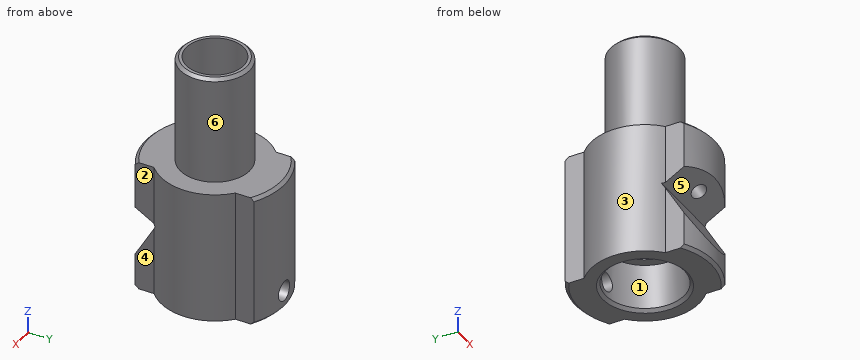
from build123d import *

# Parameters (mm, degrees)
SKETCH1_R                       = 11.5
SKETCH1_R_2                     = 4.75
BOSS_EXTRUDE1_DEPTH             = 22
SKETCH2_R                       = 5.75
SKETCH2_R_2                     = 4.75
BOSS_EXTRUDE2_DEPTH             = 18
SKETCH3_R                       = 6.5
CUT_EXTRUDE1_DEPTH              = 8
CHAMFER1_SIZE                   = 0.5
SKETCH12_W                      = 1.65
SKETCH12_H                      = 11.5
CUT_EXTRUDE4_DEPTH              = 44.179856468
CUT_EXTRUDE4_DEPTH_BACK         = 44.179856468
F_1_2_1_2_DIAMETER_HOLE1_REACH  = 40.711
F_1_2_1_2_DIAMETER_HOLE1_BORE_R = 0.6
M3_TAPPED_HOLE2_D               = 2.5
M3_TAPPED_HOLE2_DEPTH           = 4.5
M3_TAPPED_HOLE2_TIP             = 0.751075774
CHAMFER2_SIZE                   = 0.3
CHAMFER2_SIZE2                  = 8
CUT_EXTRUDE5_DEPTH              = 44.179856561
CHAMFER3_SIZE                   = 0.5


with BuildPart() as part:
    # Sketch1 → Boss-Extrude1 (new body)
    with BuildSketch(Plane.XY):
        Circle(SKETCH1_R)
        Circle(SKETCH1_R_2, mode=Mode.SUBTRACT)
    extrude(amount=BOSS_EXTRUDE1_DEPTH)

    # Sketch2 → Boss-Extrude2 (add)
    with BuildSketch(Plane.XY.offset(22)):
        Circle(SKETCH2_R)
        Circle(SKETCH2_R_2, mode=Mode.SUBTRACT)
    extrude(amount=BOSS_EXTRUDE2_DEPTH)

    # Sketch3 → Cut-Extrude1 (cut)
    with BuildSketch(Plane(origin=(0, 0, 0), x_dir=(-1, 0, 0), z_dir=(0, 0, -1))):
        Circle(SKETCH3_R)
    extrude(amount=-CUT_EXTRUDE1_DEPTH, mode=Mode.SUBTRACT)

    # Chamfer1
    chamfer1_edges = [part.edges().sort_by_distance(p)[0] for p in [
        (-11.5, 0, 0),
        (-11.5, 0, 22),
    ]]
    chamfer(chamfer1_edges, length=CHAMFER1_SIZE)

    # Sketch12 → M4 Tapped Hole3 (revolve, cut)
    with BuildSketch(Plane(origin=(0, 0, 3), x_dir=(0, 0, -1), z_dir=(1, 0, 0))):
        with Locations((0.825, 5.75)):
            Rectangle(SKETCH12_W, SKETCH12_H)
    revolve(axis=Axis((0, -6.35, 3), (0, 1, 0)), mode=Mode.SUBTRACT)

    # Sketch14 → Cut-Extrude4 (cut, two sides: drawn at the far end of the back side and taken through both)
    with BuildSketch(Plane(origin=(0, 0, 0), x_dir=(0, 0, -1), z_dir=(1, 0, 0)).offset(-CUT_EXTRUDE4_DEPTH_BACK)):
        Polygon((-15, -11.5), (-12, -6.303847577), (-3, -11.5), align=None)
    extrude(amount=CUT_EXTRUDE4_DEPTH + CUT_EXTRUDE4_DEPTH_BACK, mode=Mode.SUBTRACT)

    # Ø1.2 (1.2) Diameter Hole1 bore → Ø1.2 (1.2) Diameter Hole1 (cut, up to next)
    with BuildSketch(Plane(origin=(0, 3.620190528, 6.270353928), x_dir=(-1, 0, 0), z_dir=(0, -0.5000000000000001, -0.8660254037844386)), mode=Mode.PRIVATE) as f_1_2_1_2_diameter_hole1_sk1:
        with Locations((0, -14.459292144)):
            Circle(F_1_2_1_2_DIAMETER_HOLE1_BORE_R)
    f_1_2_1_2_diameter_hole1_tool1 = extrude(f_1_2_1_2_diameter_hole1_sk1.sketch, amount=-F_1_2_1_2_DIAMETER_HOLE1_REACH, mode=Mode.PRIVATE) & part.part
    add(f_1_2_1_2_diameter_hole1_tool1.solids().sort_by_distance((0, -8.901924, 13.5))[0], mode=Mode.SUBTRACT)

    # M3 Tapped Hole2
    with Locations(Plane(origin=(0, 3.620190528, 6.270353928), x_dir=(-1, 0, 0), z_dir=(0, -0.5000000000000001, -0.8660254037844386))):
        with Locations((0, -14.459292144)):
            Hole(M3_TAPPED_HOLE2_D / 2, depth=M3_TAPPED_HOLE2_DEPTH)
            with Locations((0, 0, -(M3_TAPPED_HOLE2_DEPTH + M3_TAPPED_HOLE2_TIP / 2))):  # 118° drill point
                Cone(0, M3_TAPPED_HOLE2_D / 2, M3_TAPPED_HOLE2_TIP, mode=Mode.SUBTRACT)

    # Chamfer2
    chamfer2_edges = [part.edges().sort_by_distance(p)[0] for p in [
        (-4.75, 0, 8),
    ]]
    chamfer2_side = [part.faces().sort_by_distance(p)[0] for p in [
        (6.316152237, 0, 8),
    ]]
    chamfer(chamfer2_edges, length=CHAMFER2_SIZE, length2=CHAMFER2_SIZE2, reference=chamfer2_side[0])

    # Sketch19 → Cut-Extrude5 (cut, through all)
    with BuildSketch(Plane(origin=(0, 0, 0), x_dir=(-1, 0, 0), z_dir=(0, 0, -1))):
        with BuildLine():
            Line((-6, 9.810708435), (-6, 6.708203932))
            ThreePointArc((-6, 6.708203932), (-9, 0), (-6, -6.708203932))
            Line((-6, -6.708203932), (-6, -9.810708435))
            ThreePointArc((-6, -9.810708435), (-11.5, 0), (-6, 9.810708435))
        make_face()
        with BuildLine():
            Line((6, 9.810708435), (6, 6.708203932))
            ThreePointArc((6, 6.708203932), (9, 0), (6, -6.708203932))
            Line((6, -6.708203932), (6, -9.810708435))
            ThreePointArc((6, -9.810708435), (11.5, 0), (6, 9.810708435))
        make_face()
    extrude(amount=-CUT_EXTRUDE5_DEPTH, mode=Mode.SUBTRACT)

    # Chamfer3
    chamfer3_edges = [part.edges().sort_by_distance(p)[0] for p in [
        (-5.75, 0, 40),
        (6.5, 0, 0),
    ]]
    chamfer(chamfer3_edges, length=CHAMFER3_SIZE)


solid = part.part
Work out the finished part from the listing and answer in its coordinate system (mm). Face numbers are marked on the shaded views. A direction names the side the tool comes from. Give positions to 0.01 mm unless a question says otherwise; leave off trailing zeros. Order: outer loops, then holes, each group sorted by start corner. A loop starts at its lowest first (then second) coordinate and runs counter-clockwise, first axis right, second up. Notation, with made-up numbers: (20, 16.25) -> (32, 16.25) arc R22 cw to (32, 32.25) -> close; hole circle Ø10 at (80.5, 81). An arc over 180 degrees is marked (long way). Answer as a JSON object with one key per item and string values. Group by question number.
1. Flat-ended cylindrical pins translate along their axes: pin 1 Ø2.5 at (y, z) = (9, 11) entering from +X; pin 2 Ø3.5 at (y, z) = (9, 7.5) entering from -X; pin 3 Ø4 at (y, z) = (-4, 13) entering from -X; pin 4 Ø8.5 at (x, y) = (0, 0) entering from +Z (3 decimals). Find the tip coordinate at first contact, or state that the pin passes through.
2. Consider line 1 along Y through (x, z) = (0, 29.25); line 2 along Z through (x, y) = (0, 8.05); line 3 along Z through (x, y) = (-2.5, -7.5). Determine where each line is inside the solid, lowest interval first. Write a range as [from, to].
3. Section B-B on z = 23 is taken. Determine the outline of the cut face in (x, y).
4. The mould has two halves that part along Y. Classify the marked faces 1, 2 and 3: released by +Y, released by -Y, zero draft, split by the parting line, or undercut.
5. A tool of negligible diameter and unlimited length cuts with its end or side. For the marked faces 4, 5 and 6, from which of +Z, -Z, +X, -X, +Y, -Y can it reach the whole face along a straight path? Write none if from no direction.
6. Section A-A on y = 0 is taken. Determine the outline of the cut face in (x, z).
7. Section C-C on x = 0 is taken. Count the separate pieces of the cut face and the enclosed holes in it, plus the area to 3 significant figures.
Result sheet:
{
 "1": {"pin 1": "stops at x = 6", "pin 2": "stops at x = -6", "pin 3": "stops at x = -8.77", "pin 4": "passes through"},
 "2": {"line 1": "y = [-5.75, -4.75], [4.75, 5.75]", "line 2": "z = [0, 1.35], [4.65, 22]", "line 3": "z = [0, 9.93], [12.69, 22]"},
 "3": {"outline": "circle Ø11.5 at (0, 0); hole circle Ø9.5 at (0, 0)"},
 "4": {"face 1": "undercut", "face 2": "zero draft", "face 3": "split by the parting line"},
 "5": {"face 4": "+Z, -Z, +X, -Y", "face 5": "+X, -X, -Y", "face 6": "+Z"},
 "6": {"outline": "(-9, 0) -> (-7, 0) -> (-6.5, 0.5) -> (-6.5, 8) -> (-5.05, 8) -> (-4.75, 16) -> (-4.75, 40) -> (-5.25, 40) -> (-5.75, 39.5) -> (-5.75, 22) -> (-9, 22) -> close; (4.75, 16) -> (5.05, 8) -> (6.5, 8) -> (6.5, 0.5) -> (7, 0) -> (9, 0) -> (9, 22) -> (5.75, 22) -> (5.75, 39.5) -> (5.25, 40) -> (4.75, 40) -> close"},
 "7": {"separate pieces": "4", "enclosed holes": "0", "area": "238 mm^2"}
}
